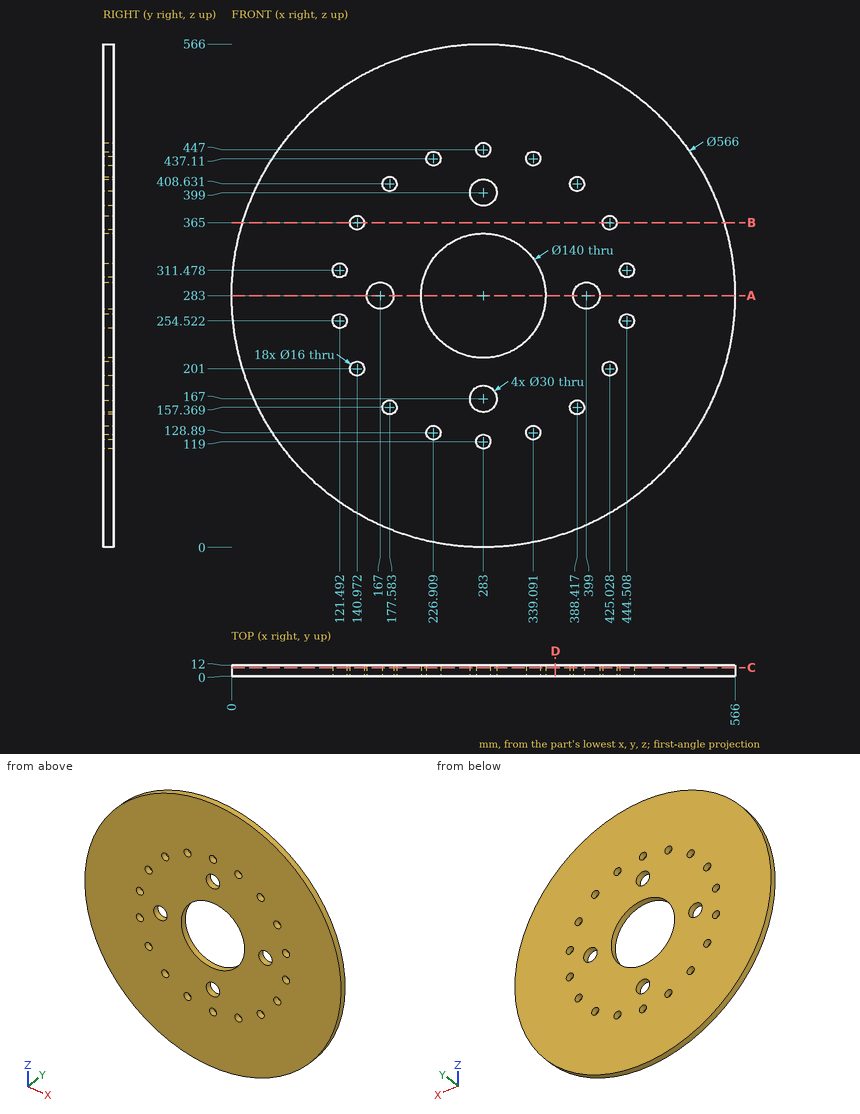
Check sheet for the drawn part. Datum: minimum x, y, z corner. Units: mm. Round coordinates to 2 decimals unless told otherwise and drop trailing zeros. Order: outer loops, then holes, each group sorted by start corner. A loop starts at its lowest first (then second) coordinate and runs counter-clockwise, first axis right, second up. Notation, with made-up numbers: M 87.5,3 L 144.5,3 A15 cw 144.5,30 Z; hole C -20,58.25 d5. An arc over 180 degrees is marked long. Write each question's results on one line, items separated by ' | '. Start each with the question number.
1. Material ranges on L1, parallel to X at y = 3, z = 201; L2, parallel to X at y = 9.75, z = 289 (1 decimal); L3, parallel to Z at x = 446.5, y = 3.75 (1 decimal), recorded low to high. Write a range as from..to.
2. Cross-section at A-A on z = 283. Record the boundary of the cut face in (x, y).
3. Go/stop test with flat-tipped pins: P1, Ø2, axis at x = 446.5, y = 6.5, coming from the +Z side (1 decimal); P2, Ø6, axis at x = 437, y = 7.5, coming from the -Z side; P3, Ø1, axis at y = 2, z = 256.5, coming from the -X side. Record where each tip stops, or that it passes through.
4. Cross-section at D-D on x = 364. Record the boundary of the cut face in (y, z).
5. Cross-section at C-C on y = 9.5. Give the number of separate pieces and of enclosed holes in the cut face, plus the area to 3 significant figures.
6. Cross-section at B-B on z = 365. Record the boundary of the cut face in (x, y).
Resolved:
1) L1: 12.14..132.97, 148.97..417.03, 433.03..553.86 | L2: 0.1..153.3, 180.7..213.3, 352.7..385.3, 412.7..565.9 | L3: 52..246.8, 262.3..303.7, 319.2..514
2) outline: M 0,0 L 152,0 L 152,12 L 0,12 Z; M 182,0 L 213,0 L 213,12 L 182,12 Z; M 353,0 L 384,0 L 384,12 L 353,12 Z; M 414,0 L 566,0 L 566,12 L 414,12 Z
3) P1: z = 514.7 | P2: z = 43.65 | P3: x = 1.2
4) outline: M 0,11.84 L 12,11.84 L 12,554.16 L 0,554.16 Z
5) separate pieces: 1 | enclosed holes: 23 | area: 230,000 mm2
6) outline: M 12.14,0 L 132.97,0 L 132.97,12 L 12.14,12 Z; M 148.97,0 L 417.03,0 L 417.03,12 L 148.97,12 Z; M 433.03,0 L 553.86,0 L 553.86,12 L 433.03,12 Z
